```python
from build123d import *

# Parameters (mm, degrees)
SKETCH1_W           = 80
SKETCH1_H           = 240
BOSS_EXTRUDE1_DEPTH = 1
SKETCH2_W           = 80
SKETCH2_H           = 1
BOSS_EXTRUDE2_DEPTH = 78
SKETCH3_W           = 80
SKETCH3_H           = 20
BOSS_EXTRUDE3_DEPTH = 1
SKETCH4_W           = 2
SKETCH4_H           = 1
CUT_EXTRUDE1_DEPTH  = 20


with BuildPart() as part:
    # Sketch1 → Boss-Extrude1 (new body)
    with BuildSketch(Plane.XY):
        Rectangle(SKETCH1_W, SKETCH1_H)
    extrude(amount=BOSS_EXTRUDE1_DEPTH)

    # Sketch2 → Boss-Extrude2 (add)
    with BuildSketch(Plane.XY.offset(1)):
        with Locations((0, 119.5)):
            Rectangle(SKETCH2_W, SKETCH2_H)
        with Locations((0, -119.5)):
            Rectangle(SKETCH2_W, SKETCH2_H)
    extrude(amount=BOSS_EXTRUDE2_DEPTH)

    # Sketch3 → Boss-Extrude3 (add)
    with BuildSketch(Plane.XY.offset(79)):
        with Locations((0, 109)):
            Rectangle(SKETCH3_W, SKETCH3_H)
    extrude(amount=-BOSS_EXTRUDE3_DEPTH)

    # Sketch4 → Cut-Extrude1 (cut)
    with BuildSketch(Plane(origin=(0, 99, 0), x_dir=(1, 0, 0), z_dir=(0, 1, 0))):
        with Locations((-39, -78.5)):
            Rectangle(SKETCH4_W, SKETCH4_H)
        with Locations((39, -78.5)):
            Rectangle(SKETCH4_W, SKETCH4_H)
    extrude(amount=CUT_EXTRUDE1_DEPTH, mode=Mode.SUBTRACT)


solid = part.part
```
The model under review builds one solid part; all positions refer to its coordinate system, in mm. A direction names the side the tool comes from. Give positions to 0.01 mm unless a question says otherwise; leave off trailing zeros. Write each loop counter-clockwise with the first axis right and the second up, starting at its lowest first coordinate (ties: lowest second). Pieces come first, ordered by that corner, then holes. Notation, with made-up numbers: M 50.25,17 L 54.25,17 A18 cw 54.25,49 Z; hole C -31.75,37.25 d1. An arc over 180 degrees is marked long. Write item = value, one per line. Start each with the question number.
Q1. Mouldability with a two-part tool opening along Z and no side actions: class faces 4 (the face through (-1, -120, 39)), 5 (the face through (-1, 119, 39)), 6 (the face through (-1, 2, 0)), 7 (the face through (-1, 110, 79)) as released by +Z, released by -Z, zero draft, split by the parting line, or undercut.
Q2. We need section B-B (x = -29.5). State the section outline as (y, z) points.
Q3. Machinability: for faces 1 (the face through (-1, -119, 39)), 2 (the face through (-1, 109, 78)), 3 (the face through (-1, 120, 39)), which of the approach directions +Z, -Z, +X, -X, +Y, -Y give a long, thin tool a straight path to every point of the face, cutting with its end or side? Answer none if there is none.
Q4. We need section A-A (z = 62). State the section outline as (x, y) points.
Q5. We need section C-C (y = 73.5). State the section outline as (x, z) points, plus the area to 3 significant figures.
Q6. Clearance check with flat-ended pins moving along their axes: pin 1 (1 mm diameter, centred on x = -3.5, y = -34.5, fed in from +Z); pin 2 (0.8 mm diameter, centred on y = 111, z = 78.5, fed in from -X). State where each tip first meets the part, or that it passes through.
Q7. For line 1 (Y direction, x = 31.5, z = 28.5); line 2 (Z direction, x = -9, y = -24), list the stretches that pass through material, from the lowest coordinate up.
Result set:
q1.face_4 = zero draft
q1.face_5 = undercut
q1.face_6 = released by -Z
q1.face_7 = released by +Z
q2.outline = M -120,0 L 120,0 L 120,79 L 99,79 L 99,78 L 119,78 L 119,1 L -119,1 L -119,79 L -120,79 Z
q3.face_1 = +Z, +X, -X
q3.face_2 = +X, -X
q3.face_3 = +Z, -Z, +X, -X, +Y
q4.outline = M -40,-120 L 40,-120 L 40,-119 L -40,-119 Z; M -40,119 L 40,119 L 40,120 L -40,120 Z
q5.outline = M -40,0 L 40,0 L 40,1 L -40,1 Z
q5.area = 80.0 mm2
q6.pin_1 = 1
q6.pin_2 = -38
q7.line_1 = -120 to -119, 119 to 120
q7.line_2 = 0 to 1
